Geometry check sheet. Reference: the model listing, model coordinates, mm. A direction names the side the tool comes from. Coordinates: 2 decimals unless noted, no trailing zeros. Loops run counter-clockwise (first coordinate to the right, second up) from the corner with the lowest first, then second, coordinate; pieces in that order, holes last.
from build123d import *

# Parameters (mm, degrees)
CAM_LOBE_DEPTH                 = 7.62
CAM_LOBE_PAIR_PATTERN_2X_COUNT = 2
CAM_LOBE_PAIR_PATTERN_2X_PITCH = 53.34
ROTATE_LOBE_180DEG_ANGLE       = 180
LOBE_SET_PATTERN_3X_COUNT      = 3
LOBE_SET_PATTERN_3X_PITCH      = 146.05
ROTATE_LOBE_SET_120DEG_ANGLE   = 120
CAMSHAFT_START                 = 49.53
SHAFT_PROFILE_SKETCH_R         = 9.5
CAMSHAFT_SHAFT_DEPTH           = 466.09


with BuildPart() as part:
    # Cam Lobe Profile Sketch → Cam Lobe (new body)
    with BuildSketch(Plane(origin=(0, 0, 0), x_dir=(1, 0, 0), z_dir=(0, 1, 0))):
        with BuildLine():
            Line((-5.499261314, 15.875), (-10.998522628, 6.35))
            ThreePointArc((-10.998522628, 6.35), (0, -12.7), (10.998522628, 6.35))
            Line((10.998522628, 6.35), (5.499261314, 15.875))
            ThreePointArc((5.499261314, 15.875), (0, 19.05), (-5.499261314, 15.875))
        make_face()
    extrude(amount=CAM_LOBE_DEPTH)


with BuildPart() as cam_lobe_pair_pattern_2x_1:
    # Cam Lobe Pair Pattern 2x: pattern copy
    add(part.part.moved(Location(Vector(0, -1, 0) * (1 * CAM_LOBE_PAIR_PATTERN_2X_PITCH))))


with BuildPart() as cam_lobe_pair_pattern_2x_1_1:
    # Rotate Lobe 180deg: moved
    add(cam_lobe_pair_pattern_2x_1.part.rotate(Axis((0, 0, 0), (0, 1, 0)), ROTATE_LOBE_180DEG_ANGLE))


with BuildPart() as lobe_set_pattern_3x_1:
    # Lobe Set Pattern 3x: pattern copy
    add(part.part.moved(Location(Vector(0, -1, 0) * (1 * LOBE_SET_PATTERN_3X_PITCH))))


with BuildPart() as lobe_set_pattern_3x_2:
    # Lobe Set Pattern 3x: pattern copy
    add(part.part.moved(Location(Vector(0, -1, 0) * (2 * LOBE_SET_PATTERN_3X_PITCH))))


with BuildPart() as lobe_set_pattern_3x_3:
    # Lobe Set Pattern 3x: pattern copy
    add(cam_lobe_pair_pattern_2x_1_1.part.moved(Location(Vector(0, -1, 0) * (1 * LOBE_SET_PATTERN_3X_PITCH))))


with BuildPart() as lobe_set_pattern_3x_4:
    # Lobe Set Pattern 3x: pattern copy
    add(cam_lobe_pair_pattern_2x_1_1.part.moved(Location(Vector(0, -1, 0) * (2 * LOBE_SET_PATTERN_3X_PITCH))))


with BuildPart() as lobe_set_pattern_3x_1_1:
    # Rotate Lobe Set 120deg: moved
    add(lobe_set_pattern_3x_1.part.rotate(Axis((0, 0, 0), (0, -1, 0)), ROTATE_LOBE_SET_120DEG_ANGLE))


with BuildPart() as lobe_set_pattern_3x_3_1:
    # Rotate Lobe Set 120deg: moved
    add(lobe_set_pattern_3x_3.part.rotate(Axis((0, 0, 0), (0, -1, 0)), ROTATE_LOBE_SET_120DEG_ANGLE))


with BuildPart() as part_1:
    add(part.part)

    add(cam_lobe_pair_pattern_2x_1_1.part)  # Camshaft Shaft merges Cam Lobe Pair Pattern 2x_1

    add(lobe_set_pattern_3x_1_1.part)  # Camshaft Shaft merges Lobe Set Pattern 3x_1

    add(lobe_set_pattern_3x_2.part)  # Camshaft Shaft merges Lobe Set Pattern 3x_2

    add(lobe_set_pattern_3x_3_1.part)  # Camshaft Shaft merges Lobe Set Pattern 3x_3

    add(lobe_set_pattern_3x_4.part)  # Camshaft Shaft merges Lobe Set Pattern 3x_4
    # Shaft Profile Sketch → Camshaft Shaft (add)
    with BuildSketch(Plane(origin=(0, 0, 0), x_dir=(1, 0, 0), z_dir=(0, 1, 0)).offset(CAMSHAFT_START)):
        with Locations(Location((0, 0, 0), (0, 0, 270))):
            Circle(SHAFT_PROFILE_SKETCH_R)
    extrude(amount=-CAMSHAFT_SHAFT_DEPTH)


solid = part_1.part
(1) Gauge pin test, flat ends, axial feed: pin 1 Ø2 at (x, y) = (-1, -256.5) entering from +Z; pin 2 Ø3 at (y, z) = (-355, 5.5) entering from +X; pin 3 Ø6 at (y, z) = (-308, -7.5) entering from -X. Record the tip position at first contact, or that the pin passes through.
Findings:
pin 1: stops at z = 9.5
pin 2: stops at x = 8.62
pin 3: stops at x = -8.37
(2) Sectioned sample at A-A on y = -96. Record the cut outline in (x, z), and give its area (3 significant figures).
Findings:
outline: circle Ø19 at (0, 0)
area: 284 mm2
(3) Scan lines: L1, parallel to Y at x = -6.5, z = 8; L2, parallel to Y at x = -1, z = -17; L3, parallel to Y at x = -0.5, z = 17. Record each from-to range of solid material in increasing order.
Findings:
L1: y = -345.44 to -337.82, -292.1 to -284.48, -199.39 to -191.77, -146.05 to -138.43, -53.34 to -45.72, 0 to 7.62
L2: y = -292.1 to -284.48, 0 to 7.62
L3: y = -345.44 to -337.82, -53.34 to -45.72
(4) Access from +Z, -Z, +X, -X, +Y, -Y to the whole of each face (thin tool, end or side, straight path). Record for faces 1 (the flat face through (5, -142, 12.7)), 2 (the cylindrical face through (-5.78, -380.5, -7.54)), 3 (the flat face through (1, 7.62, -10)), 4 (the cylindrical face through (-5.78, -241.34, -7.54)), 5 (the flat face through (-5, -196, -12.7)).
Findings:
face 1: +Z, +X, -X
face 2: -Y
face 3: +Y
face 4: none
face 5: -Z, +X, -X
(5) Draft check along Y on faces 6 (the flat face through (8.2, -341.7, 11.2)), 7 (the flat face through (-1, -53.34, 10)), 8 (the cylindrical face through (0.372, -49.583, -12.695)), 9 (the flat face through (0, 49.53, 0)). Enter one of: +Y half, -Y half, draft (parallel to the pull), parting line (faces both ways), or undercut.
Findings:
face 6: draft
face 7: undercut
face 8: undercut
face 9: +Y half
